Here's the drawing with two shaded views (mm, measured from the low corner). I have some questions. A direction names the side the tool comes from. Give positions to 0.01 mm unless a question says otherwise; leave off trailing zeros. Loops run counter-clockwise (first coordinate to the right, second up) from the corner with the lowest first, then second, coordinate; pieces in that order, holes last. Notation, with made-up numbers: (13, 54) - (43, 54) arc R35 ccw to (43, 88) - close; hole circle Ø3 at (73, 69). An arc over 180 degrees is marked (long way). Answer as a JSON object with one key per item and string values. Group by question number.
Item 1: Suppose I cut it at A-A on y = 5.75. Write out the boundary of the cut face in (x, z).
Item 2: Which directions (+Z, -Z, +X, -X, +Y, -Y) give clear straight access to the entire face, cutting with the end or side of a thin tool? Please do the marked faces 4 and 5.
Item 3: Suppose I cut it at B-B on x = 4. Write out the boundary of the cut face in (y, z).
Item 4: Please list where these lines run through material, in increasing order: L1, parallel to X at y = 15.75, z = 41.4; L2, parallel to X at y = 5.75, z = 18; L3, parallel to Y at x = 10.5, z = 39.
Item 5: Suppose I cut it at C-C on z = 41.4. Write out the boundary of the cut face in (x, y), and give its area (3 significant figures).
Item 6: Thinking about a two-plate mould opening in X: for the marked faces 1, 2 and 3, which applies, pulls with the +X half, pulls with the -X half, needs draft (parallel to the pull), parting line crosses it, or undercut?
Item 7: Suppose I cut it at D-D on z = 29. Write out the boundary of the cut face in (x, y).
Item 8: Will these pins go through, and if not, where does the flat tip stop? pin 1 (1.1 mm diameter, centred on x = 3.5, z = 41.5, fed in from +Y); pin 2 (10 mm diameter, centred on x = 19, z = 8.5, fed in from -Y).
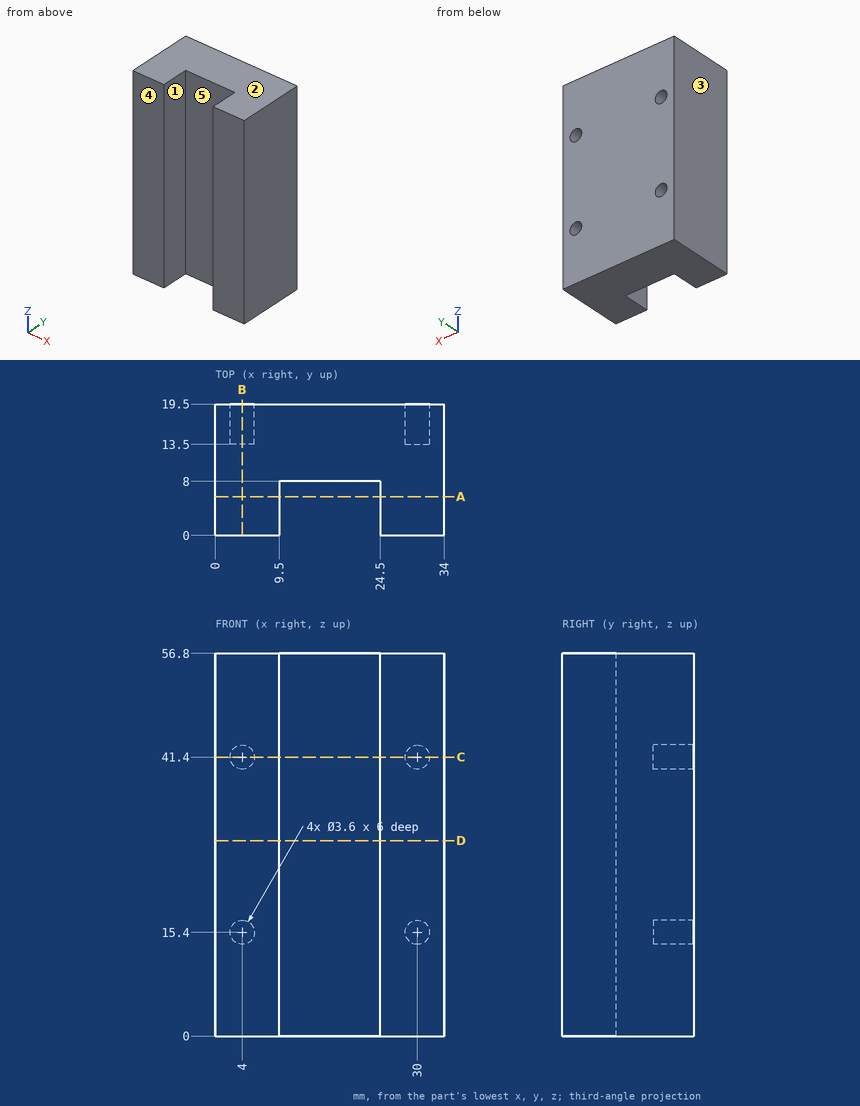
Worked out:
{
 "1": {"outline": "(0, 0) - (9.5, 0) - (9.5, 56.8) - (0, 56.8) - close; (24.5, 0) - (34, 0) - (34, 56.8) - (24.5, 56.8) - close"},
 "2": {"face 4": "+Z, -Z, +X, -X, -Y", "face 5": "+Z, -Z, -Y"},
 "3": {"outline": "(0, 0) - (19.5, 0) - (19.5, 13.6) - (13.5, 13.6) - (13.5, 17.2) - (19.5, 17.2) - (19.5, 39.6) - (13.5, 39.6) - (13.5, 43.2) - (19.5, 43.2) - (19.5, 56.8) - (0, 56.8) - close"},
 "4": {"L1": "x = 0 to 2.2, 5.8 to 28.2, 31.8 to 34", "L2": "x = 0 to 9.5, 24.5 to 34", "L3": "y = 8 to 19.5"},
 "5": {"outline": "(0, 0) - (9.5, 0) - (9.5, 8) - (24.5, 8) - (24.5, 0) - (34, 0) - (34, 19.5) - (31.8, 19.5) - (31.8, 13.5) - (28.2, 13.5) - (28.2, 19.5) - (5.8, 19.5) - (5.8, 13.5) - (2.2, 13.5) - (2.2, 19.5) - (0, 19.5) - close", "area": "500 mm2"},
 "6": {"face 1": "undercut", "face 2": "needs draft", "face 3": "pulls with the -X half"},
 "7": {"outline": "(0, 0) - (9.5, 0) - (9.5, 8) - (24.5, 8) - (24.5, 0) - (34, 0) - (34, 19.5) - (0, 19.5) - close"},
 "8": {"pin 1": "stops at y = 13.5", "pin 2": "stops at y = 8"}
}
